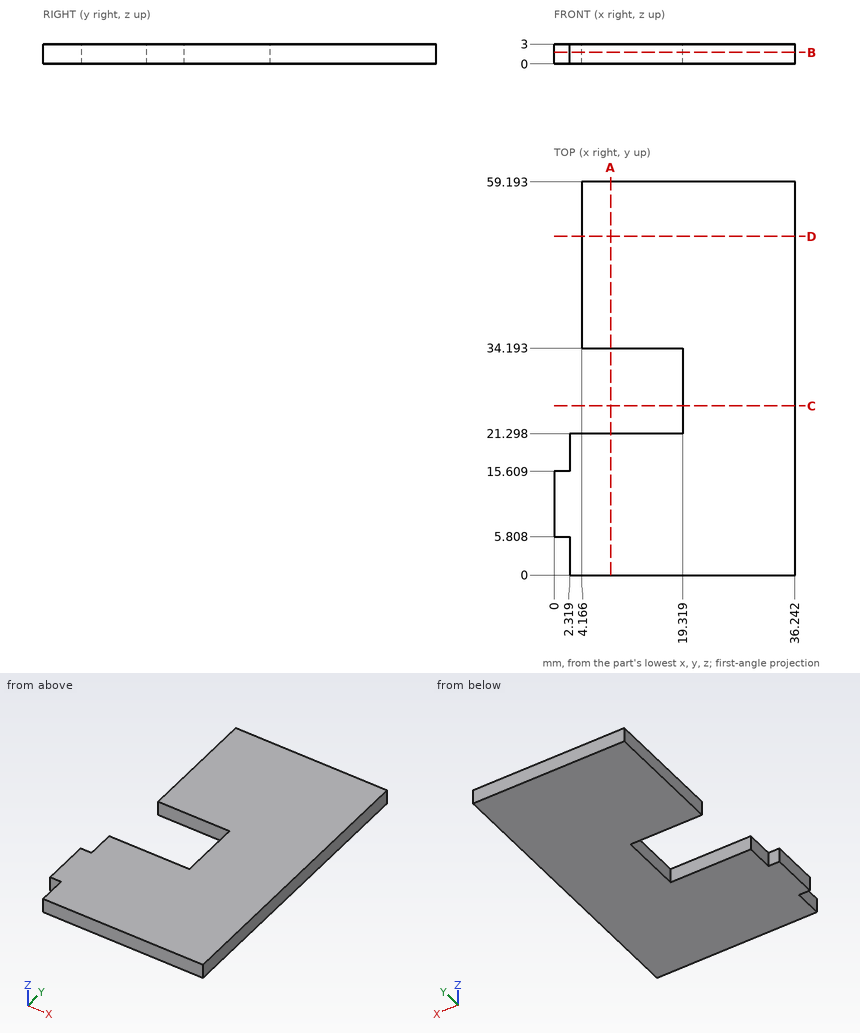
Drawing for the job (mm, zero at the part's lowest x, y, z). Give positions to 0.01 mm unless a question says otherwise; leave off trailing zeros. Order: outer loops, then holes, each group sorted by start corner. A loop starts at its lowest first (then second) coordinate and runs counter-clockwise, first axis right, second up. Notation, with made-up numbers: M 33.5,-16 L 79.5,-16 A19 ccw 79.5,12 Z; hole C 40,12 d8. An arc over 180 degrees is marked long. Use a Markdown table: item, result. Add a question column.
(1) Saw through at D-D, the plane y = 51. Give the cut face in (x, z).
(2) Probe line 1 along Y through (x, z) = (16, 1.3); line 2 along X through (y, z) = (56, 1.3); line 3 along X through (y, z) = (16, 0.5). List the from-to ranges inside material, lowest first. Write a range as [from, to].
(3) Drop flat-ended pins along their axis: P1, Ø1.5, axis at y = 24.5, z = 1, coming from the -X side; P2, Ø1.5, axis at y = 2.5, z = 2, coming from the -X side; P3, Ø5, axis at x = 15.5, y = 7, coming from the -Z side. Give the stop position or say it passes through.
(4) Saw through at C-C, the plane y = 25.5. Give the cut face in (x, z).
(5) Saw through at A-A, the plane x = 8.5. Give the cut face in (y, z), and give its area (3 significant figures).
(6) Saw through at B-B, the plane z = 1.75. Give the cut face in (x, y).
Answer key:
| question | item | result |
|---|---|---|
| 1 | outline | M 4.17,0 L 36.24,0 L 36.24,3 L 4.17,3 Z |
| 2 | line 1 | [0, 21.3], [34.19, 59.19] |
| 2 | line 2 | [4.17, 36.24] |
| 2 | line 3 | [2.32, 36.24] |
| 3 | P1 | x = 19.32 |
| 3 | P2 | x = 2.32 |
| 3 | P3 | z = 0 |
| 4 | outline | M 19.32,0 L 36.24,0 L 36.24,3 L 19.32,3 Z |
| 5 | outline | M 0,0 L 21.3,0 L 21.3,3 L 0,3 Z; M 34.19,0 L 59.19,0 L 59.19,3 L 34.19,3 Z |
| 5 | area | 139 mm^2 |
| 6 | outline | M 0,5.81 L 2.32,5.81 L 2.32,0 L 36.24,0 L 36.24,59.19 L 4.17,59.19 L 4.17,34.19 L 19.32,34.19 L 19.32,21.3 L 2.32,21.3 L 2.32,15.61 L 0,15.61 Z |
